from build123d import *

# Parameters (mm, degrees)
SKETCH_1_W          = 80
SKETCH_1_H          = 60
EXTRUDE_1_DEPTH     = 20
CUT_EXTRUDE_1_REACH = 55.852
SKETCH_2_W          = 48
SKETCH_2_H          = 50
SKETCH_3_W          = 60
SKETCH_3_H          = 50
CUT_EXTRUDE_2_DEPTH = 14


with BuildPart() as part:
    # 草图1 → 凸台-拉伸1 (new body)
    with BuildSketch(Plane.XY):
        Rectangle(SKETCH_1_W, SKETCH_1_H)
    extrude(amount=EXTRUDE_1_DEPTH)

    # 草图2 → 切除-拉伸1 (cut, up to next)
    with BuildSketch(Plane.XY.offset(20), mode=Mode.PRIVATE) as cut_extrude_1_sk1:
        Rectangle(SKETCH_2_W, SKETCH_2_H)
    cut_extrude_1_tool1 = extrude(cut_extrude_1_sk1.sketch, amount=-CUT_EXTRUDE_1_REACH, mode=Mode.PRIVATE) & part.part
    add(cut_extrude_1_tool1.solids().sort_by_distance((0, 0, 20))[0], mode=Mode.SUBTRACT)

    # 草图3 → 切除-拉伸2 (cut)
    with BuildSketch(Plane(origin=(0, 0, 0), x_dir=(-1, 0, 0), z_dir=(0, 0, -1))):
        Rectangle(SKETCH_3_W, SKETCH_3_H)
    extrude(amount=-CUT_EXTRUDE_2_DEPTH, mode=Mode.SUBTRACT)


solid = part.part
For this review, take the finished solid that the model builds, in its own axes (mm). A direction names the side the tool comes from. Give positions to 0.01 mm unless a question says otherwise; leave off trailing zeros. Loops run counter-clockwise (first coordinate to the right, second up) from the corner with the lowest first, then second, coordinate; pieces in that order, holes last.
Item 1: Insertion check: pin 1 (8 mm diameter, centred on x = 19.5, y = -8, fed in from +Z); pin 2 (1.8 mm diameter, centred on x = 27.5, y = -1.5, fed in from -Z). Each pin has a flat end and moves straight along its axis. Give the tip position at first contact, or say it passes through.
Item 2: Take a section at B-B, the plane y = 3. State the section outline as (x, z) points, and give its area (3 significant figures).
Item 3: Take a section at A-A, the plane x = -21. State the section outline as (y, z) points, and give its area (3 significant figures).
Item 4: Take a section at C-C, the plane z = 16.5. State the section outline as (x, y) points.
Item 5: For line 1 along Y through (x, z) = (29.5, 6.5); line 2 along X through (y, z) = (22.5, 5.25); line 3 along X through (y, z) = (-8, 15.5), list the stretches that pass through material, from the lowest coordinate up.
Item 6: Tool access review of faces 5 (the flat face through (24, 0, 17)), 6 (the flat face through (-30, 0, 7)), 7 (the flat face through (-27, 0, 20)): name each direction out of +Z, -Z, +X, -X, +Y, -Y from which nothing blocks a thin tool from reaching the whole face with its end or side.
Item 7: Draft analysis for pull direction Y (two halves, no side actions). For faces 1 (the flat face through (-1, -30, 10)), 2 (the flat face through (-1, -26, 0)), 3 (the flat face through (0, -25, 10)), 4 (the flat face through (30, 0, 7)), state which applies: +Y half, -Y half, draft (parallel to the pull), parting line (faces both ways), or undercut.
Item 8: Take a section at D-D, the plane x = -29. State the section outline as (y, z) points.
Calculated:
1. pin 1: passes through
1. pin 2: stops at z = 14
2. outline: (-40, 0) - (-30, 0) - (-30, 14) - (-24, 14) - (-24, 20) - (-40, 20) - close; (24, 14) - (30, 14) - (30, 0) - (40, 0) - (40, 20) - (24, 20) - close
2. area: 472 mm2
3. outline: (-30, 0) - (-25, 0) - (-25, 20) - (-30, 20) - close; (25, 0) - (30, 0) - (30, 20) - (25, 20) - close
3. area: 200 mm2
4. outline: (-40, -30) - (40, -30) - (40, 30) - (-40, 30) - close; hole (-24, -25) - (24, -25) - (24, 25) - (-24, 25) - close
5. line 1: y = -30 to -25, 25 to 30
5. line 2: x = -40 to -30, 30 to 40
5. line 3: x = -40 to -24, 24 to 40
6. face 5: +Z, -Z
6. face 6: -Z
6. face 7: +Z, +X, -X, +Y, -Y
7. face 1: -Y half
7. face 2: draft
7. face 3: undercut
7. face 4: undercut
8. outline: (-30, 0) - (-25, 0) - (-25, 14) - (25, 14) - (25, 0) - (30, 0) - (30, 20) - (-30, 20) - close
